from build123d import *

# Parameters (mm, degrees)
SKETCH_1_R             = 4.25
EXTRUDE_1_DEPTH        = 1.5
SKETCH_2_R             = 2
EXTRUDE_2_DEPTH        = 10
HOLE_WIZARD_M3_1_D     = 2.5
HOLE_WIZARD_M3_1_DEPTH = 8.5
HOLE_WIZARD_M3_1_TIP   = 0.751075774
CUT_EXTRUDE_1_DEPTH    = 1
CHAMFER_1_SIZE         = 0.5
CHAMFER_2_SIZE         = 0.1


with BuildPart() as part:
    # 草图1 → 凸台-拉伸1 (new body)
    with BuildSketch(Plane(origin=(0, 0, 0), x_dir=(1, 0, 0), z_dir=(0, 1, 0))):
        with Locations(Location((0, 0, 0), (0, 0, 270))):
            Circle(SKETCH_1_R)
    extrude(amount=EXTRUDE_1_DEPTH)

    # 草图2 → 凸台-拉伸2 (add)
    with BuildSketch(Plane(origin=(0, 1.5, 0), x_dir=(1, 0, 0), z_dir=(0, 1, 0))):
        with Locations(Location((0, 0, 0), (0, 0, 270))):
            Circle(SKETCH_2_R)
    extrude(amount=EXTRUDE_2_DEPTH)

    # M3 螺纹孔1
    with Locations(Plane(origin=(0, 11.5, 0), x_dir=(1, 0, 0), z_dir=(0, 1, 0))):
        with Locations((0, 0)):
            Hole(HOLE_WIZARD_M3_1_D / 2, depth=HOLE_WIZARD_M3_1_DEPTH)
            with Locations((0, 0, -(HOLE_WIZARD_M3_1_DEPTH + HOLE_WIZARD_M3_1_TIP / 2))):  # 118° drill point
                Cone(0, HOLE_WIZARD_M3_1_D / 2, HOLE_WIZARD_M3_1_TIP, mode=Mode.SUBTRACT)

    # 草图7 → 切除-拉伸1 (cut)
    with BuildSketch(Plane.XZ):
        Polygon((0, 1.443375673), (-1.25, 0.721687836), (-1.25, -0.721687836), (0, -1.443375673), (1.25, -0.721687836), (1.25, 0.721687836), align=None)
    extrude(amount=-CUT_EXTRUDE_1_DEPTH, mode=Mode.SUBTRACT)

    # 倒角1
    chamfer_1_edges = [part.edges().sort_by_distance(p)[0] for p in [
        (0, 0, -4.25),
    ]]
    chamfer(chamfer_1_edges, length=CHAMFER_1_SIZE)

    # 倒角2
    chamfer_2_edges = [part.edges().sort_by_distance(p)[0] for p in [
        (0, 1.5, -4.25),
    ]]
    chamfer(chamfer_2_edges, length=CHAMFER_2_SIZE)


solid = part.part
Can you work these out from the model? Positions are in its coordinate system, mm. A direction names the side the tool comes from. Give positions to 0.01 mm unless a question says otherwise; leave off trailing zeros. Write each loop counter-clockwise with the first axis right and the second up, starting at its lowest first coordinate (ties: lowest second). Pieces come first, ordered by that corner, then holes. Notation, with made-up numbers: (9.5, 74.25) -> (30.5, 74.25) arc R25 cw to (30.5, 113.25) -> close; hole circle Ø11 at (49, 45.5). An arc over 180 degrees is marked (long way). Answer as a JSON object with one key per item and string values. Group by question number.
Item 1: I'm going to push flat-ended pins straight in: P1, Ø5, axis at x = 3, z = 0.5, coming from the -Y side; P2, Ø2, axis at x = -3.5, z = 0.5, coming from the +Y side; P3, Ø5, axis at y = 5.5, z = -1.5, coming from the +X side; P4, Ø2, axis at x = 0, z = 0, coming from the -Y side. Where does each tip first touch, or does it pass through?
Item 2: Please list where these lines run through material, in increasing order: line 1 (Y direction, x = -2, z = -1.5); line 2 (X direction, y = 9, z = -0.25); line 3 (Z direction, x = 0.5, y = 6.25). Write a range as [from, to].
Item 3: For faces 1 (the face through (1, 11.5, 1)), 2 (the face through (1, 1.5, 2)), 3 (the face through (-1.25, 0.5, 0)), which set-ups out of +Z, -Z, +X, -X, +Y, -Y let a thin tool reach every point of the face, with its end or its side?
Item 4: We'd pull the mould along X, two halves only. Please class faces 4 (the face through (-2, 0, 0)), 5 (the face through (0, 1, 0)), 6 (the face through (4.214, 0.944, -0.553)), 7 (the face through (0.616, 0.493, -1.088)): +X half, -X half, draft (parallel to the pull), parting line (faces both ways), or undercut.
Item 5: Suppose I cut it at A-A (y = 4). Please give me the cut outline in (x, z), plus the area to 3 significant figures.
Item 6: Suppose I cut it at B-B (y = 1.25). Please give me the cut outline in (x, z), plus the area to 3 significant figures.
Findings:
{
 "1": {"P1": "stops at y = 0", "P2": "stops at y = 1.5", "P3": "stops at x = 2", "P4": "stops at y = 1"},
 "2": {"line 1": "y = [0, 1.5]", "line 2": "x = [-1.98, -1.22], [1.22, 1.98]", "line 3": "z = [-1.94, -1.15], [1.15, 1.94]"},
 "3": {"face 1": "+Z, -Z, +X, -X, +Y", "face 2": "+Y", "face 3": "-Y"},
 "4": {"face 4": "draft", "face 5": "undercut", "face 6": "parting line", "face 7": "undercut"},
 "5": {"outline": "circle Ø4 at (0, 0); hole circle Ø2.5 at (0, 0)", "area": "7.66 mm²"},
 "6": {"outline": "circle Ø8.5 at (0, 0)", "area": "56.7 mm²"}
}
